Source: CAD feature listing. Evaluate the final solid. Frame: model axes, mm. A direction names the side the tool comes from. Coordinates: 2 decimals unless noted, no trailing zeros. Order: outer loops, then holes, each group sorted by start corner. A loop starts at its lowest first (then second) coordinate and runs counter-clockwise, first axis right, second up.
```python
from build123d import *

# Parameters (mm, degrees)
SKETCH1_W           = 42
SKETCH1_H           = 42
SKETCH1_R           = 1.5
BOSS_EXTRUDE1_DEPTH = 47
CUT_EXTRUDE1_DEPTH  = 56.596762496
SKETCH4_R           = 11
BOSS_EXTRUDE2_DEPTH = 2
BOSS_EXTRUDE3_DEPTH = 20
CUT_EXTRUDE2_DEPTH  = 2
SKETCH8_R           = 3
CUT_EXTRUDE3_DEPTH  = 2
BOSS_EXTRUDE4_START = 1.9
SKETCH9_R           = 2.5
BOSS_EXTRUDE4_DEPTH = 1.9
SKETCH10_W          = 3
SKETCH10_H          = 10.31009041
SKETCH10_W_2        = 2.478607588
SKETCH10_H_2        = 8.518222776
BOSS_EXTRUDE5_DEPTH = 5
SKETCH11_R          = 0.5
BOSS_EXTRUDE6_DEPTH = 5


with BuildPart() as part:
    # Sketch1 → Boss-Extrude1 (new body)
    with BuildSketch(Plane.XY):
        Rectangle(SKETCH1_W, SKETCH1_H)
        with Locations((-15.5, 15.5)):
            Circle(SKETCH1_R, mode=Mode.SUBTRACT)
        with Locations(Location((15.5, 15.5, 0), (0, 0, 180))):
            Circle(SKETCH1_R, mode=Mode.SUBTRACT)
        with Locations(Location((-15.5, -15.5, 0), (0, 0, 180))):
            Circle(SKETCH1_R, mode=Mode.SUBTRACT)
        with Locations((15.5, -15.5)):
            Circle(SKETCH1_R, mode=Mode.SUBTRACT)
    extrude(amount=BOSS_EXTRUDE1_DEPTH)

    # Sketch3 → Cut-Extrude1 (cut, through all)
    with BuildSketch(Plane(origin=(0, 0, 0), x_dir=(-1, 0, 0), z_dir=(0, 0, -1))):
        Polygon((-21, 17), (-17, 21), (-21, 21), align=None)
        Polygon((21, 21), (17, 21), (21, 17), align=None)
        Polygon((21, -17), (17, -21), (21, -21), align=None)
        Polygon((-21, -21), (-17, -21), (-21, -17), align=None)
    extrude(amount=-CUT_EXTRUDE1_DEPTH, mode=Mode.SUBTRACT)

    # Sketch4 → Boss-Extrude2 (add)
    with BuildSketch(Plane(origin=(0, 0, 0), x_dir=(-1, 0, 0), z_dir=(0, 0, -1))):
        Circle(SKETCH4_R)
    extrude(amount=BOSS_EXTRUDE2_DEPTH)

    # Sketch5 → Boss-Extrude3 (add)
    with BuildSketch(Plane(origin=(0, 0, -2), x_dir=(-1, 0, 0), z_dir=(0, 0, -1))):
        with BuildLine():
            Line((1.7, -1.833030278), (1.7, 1.833030278))
            ThreePointArc((1.7, 1.833030278), (-2.5, 0), (1.7, -1.833030278))
        make_face()
    extrude(amount=BOSS_EXTRUDE3_DEPTH)

    # Sketch7 → Cut-Extrude2 (cut)
    with BuildSketch(Plane.XY.offset(47)):
        with BuildLine():
            Line((21, 17), (21, 11.625484678))
            ThreePointArc((21, 11.625484678), (13.597062084, 13.597062084), (11.625484678, 21))
            Line((11.625484678, 21), (17, 21))
            Line((17, 21), (21, 17))
        make_face()
        with BuildLine():
            Line((-21, -17), (-21, -11.625484678))
            ThreePointArc((-21, -11.625484678), (-13.597062084, -13.597062084), (-11.625484678, -21))
            Line((-11.625484678, -21), (-17, -21))
            Line((-17, -21), (-21, -17))
        make_face()
        with BuildLine():
            Line((-11.625484678, 21), (-17, 21))
            Line((-17, 21), (-21, 17))
            Line((-21, 17), (-21, 11.625484678))
            ThreePointArc((-21, 11.625484678), (-13.597062084, 13.597062084), (-11.625484678, 21))
        make_face()
        with BuildLine():
            Line((11.625484678, -21), (17, -21))
            Line((17, -21), (21, -17))
            Line((21, -17), (21, -11.625484678))
            ThreePointArc((21, -11.625484678), (13.597062084, -13.597062084), (11.625484678, -21))
        make_face()
    extrude(amount=-CUT_EXTRUDE2_DEPTH, mode=Mode.SUBTRACT)

    # Sketch8 → Cut-Extrude3 (cut)
    with BuildSketch(Plane.XY.offset(47)):
        Circle(SKETCH8_R)
    extrude(amount=-CUT_EXTRUDE3_DEPTH, mode=Mode.SUBTRACT)

    # Sketch9 → Boss-Extrude4 (add)
    with BuildSketch(Plane.XY.offset(45).offset(BOSS_EXTRUDE4_START)):
        with Locations(Location((0, 0, 0), (0, 0, 180))):
            Circle(SKETCH9_R)
    extrude(amount=-BOSS_EXTRUDE4_DEPTH)

    # Sketch10 → Boss-Extrude5 (add)
    with BuildSketch(Plane.ZY.offset(21)):
        with Locations((45.5, 0)):
            Rectangle(SKETCH10_W, SKETCH10_H)
        with Locations((45.5, 0)):
            Rectangle(SKETCH10_W_2, SKETCH10_H_2, mode=Mode.SUBTRACT)
    extrude(amount=BOSS_EXTRUDE5_DEPTH)

    # Sketch11 → Boss-Extrude6 (add)
    with BuildSketch(Plane.ZY.offset(21)):
        with Locations(Location((45.5, 3.127782029, 0), (0, 0, 180))):
            Circle(SKETCH11_R)
        with Locations(Location((45.5, 1.627782029, 0), (0, 0, 180))):
            Circle(SKETCH11_R)
        with Locations(Location((45.5, 0.127782029, 0), (0, 0, 180))):
            Circle(SKETCH11_R)
        with Locations(Location((45.5, -1.372217971, 0), (0, 0, 180))):
            Circle(SKETCH11_R)
        with Locations(Location((45.5, -2.872217971, 0), (0, 0, 180))):
            Circle(SKETCH11_R)
    extrude(amount=BOSS_EXTRUDE6_DEPTH)


solid = part.part
```
Q1. Section query D-D on x = -10. Output: boundary loops of the cut face in (y, z).
Solutions:
outline: (-21, 0) - (-4.58, 0) - (-4.58, -2) - (4.58, -2) - (4.58, 0) - (21, 0) - (21, 47) - (-21, 47) - close
Q2. Material intervals for line 1 along X through (y, z) = (-15.5, 23); line 2 along Y through (x, z) = (15, 36), sorted ascending.
Solutions:
line 1: x = -21 to -17, -14 to 14, 17 to 21
line 2: y = -21 to -16.91, -14.09 to 14.09, 16.91 to 21
Q3. Set-up query: faces 5 (the flat face through (-23, -5.155, 45)), 6 (the cylindrical face through (13.677, 13.518, 46.014)), 7 (the flat face through (-21, -0.1, 44.7)), 8 (the flat face through (-23, 0, 44)). Return all of +Z, -Z, +X, -X, +Y, -Y with unobstructed straight access to the full face (end or side cutting, diameter ignored); none if empty.
Solutions:
face 5: +Z, -Z, -X, -Y
face 6: +Z
face 7: -X
face 8: -Z, -X, +Y, -Y
Q4. Pin query (flat end, axial travel): P1, Ø1.8, axis at y = -0.5, z = -10.5, coming from the -X side; P2, Ø8, axis at y = -9, z = -12.5, coming from the -X side; P3, Ø3, axis at x = 0.5, y = -0.5, coming from the +Z side; P4, Ø4, axis at x = -24, y = 1.5, coming from the -Z side. Return the tip coordinate at first contact, or that it passes through.
Solutions:
P1: stops at x = -1.7
P2: passes through
P3: stops at z = 46.9
P4: stops at z = 44
Q5. Section query A-A on z = 21. Output: boundary loops of the cut face in (x, y), plus the area to 3 significant figures.
Solutions:
outline: (-21, -17) - (-17, -21) - (17, -21) - (21, -17) - (21, 17) - (17, 21) - (-17, 21) - (-21, 17) - close; hole circle Ø3 at (-15.5, -15.5); hole circle Ø3 at (-15.5, 15.5); hole circle Ø3 at (15.5, -15.5); hole circle Ø3 at (15.5, 15.5)
area: 1,700 mm2
Q6. Pull-direction query (X, two-part tool) for faces 1 (the flat face through (19, 19, 22)), 2 (the flat face through (-23, 4.259, 45)), 3 (the flat face through (-2, 2, 45)), 4 (the cylindrical face through (-17, 15.57, 22.18)); classes: pulls with the +X half, pulls with the -X half, needs draft (parallel to the pull), parting line crosses it, or undercut.
Solutions:
face 1: pulls with the +X half
face 2: needs draft
face 3: undercut
face 4: undercut
Q7. Section query B-B on y = 15.5. Output: boundary loops of the cut face in (x, z), plus the area to 3 significant figures.
Solutions:
outline: (-21, 0) - (-17, 0) - (-17, 45) - (-21, 45) - close; (-14, 0) - (14, 0) - (14, 45) - (12.21, 45) - (12.21, 47) - (-12.21, 47) - (-12.21, 45) - (-14, 45) - close; (17, 0) - (21, 0) - (21, 45) - (17, 45) - close
area: 1,670 mm2
